from build123d import *

# Parameters (mm, degrees)
FORK_BOSS_15MM_DEPTH           = 15
SKETCH1_10_R                   = 11.5
SKETCH1_10_R_2                 = 4.5
PLATE_BOSS_12MM_DEPTH          = 12
POCKET_START                   = -7
POCKET_AND_HOLES_CUT_7MM_DEPTH = 7


with BuildPart() as part:
    # Bracket Outline Sketch → Fork Boss 15mm (new body)
    with BuildSketch(Plane.XY):
        with BuildLine():
            Line((-17.348851567, 85.016364122), (17.292164585, 65.016364122))
            ThreePointArc((17.292164585, 65.016364122), (21.08625981, 64.51686201), (24.122291604, 66.846491141))
            Line((24.122291604, 66.846491141), (29.979005279, 76.990616791))
            Line((29.979005279, 76.990616791), (39.122291604, 92.827253255))
            Line((39.122291604, 92.827253255), (30.490381057, 97.810889132))
            Line((30.490381057, 97.810889132), (17.990381057, 76.160254038))
            Line((17.990381057, 76.160254038), (-7.990381057, 91.160254038))
            Line((-7.990381057, 91.160254038), (4.509618943, 112.810889132))
            Line((4.509618943, 112.810889132), (-4.178978585, 117.827253255))
            Line((-4.178978585, 117.827253255), (-19.178978585, 91.846491141))
            ThreePointArc((-19.178978585, 91.846491141), (-19.678480698, 88.052395915), (-17.348851567, 85.016364122))
        make_face()
    extrude(amount=FORK_BOSS_15MM_DEPTH)

    # Sketch1_10 → Plate Boss 12mm (add)
    with BuildSketch(Plane.XY):
        with BuildLine():
            ThreePointArc((24.122291604, 66.846491141), (21.08625981, 64.51686201), (17.292164585, 65.016364122))
            Line((17.292164585, 65.016364122), (-17.348851567, 85.016364122))
            ThreePointArc((-17.348851567, 85.016364122), (-19.678480698, 88.052395915), (-19.178978585, 91.846491141))
            Line((-19.178978585, 91.846491141), (-22.741186866, 85.676565412))
            ThreePointArc((-22.741186866, 85.676565412), (-25.323096431, 80.149782404), (-26.906195607, 74.258654802))
            Line((-26.906195607, 74.258654802), (-38.965270802, 5.868240888))
            ThreePointArc((-38.965270802, 5.868240888), (-37.871454253, 1.786061952), (-34.041232037, 0))
            Line((-34.041232037, 0), (34.041232037, 0))
            ThreePointArc((34.041232037, 0), (37.871454253, 1.786061952), (38.965270802, 5.868240888))
            Line((38.965270802, 5.868240888), (28.201741138, 66.911250985))
            ThreePointArc((28.201741138, 66.911250985), (28.201741138, 72.107623698), (29.979005279, 76.990616791))
            Line((29.979005279, 76.990616791), (24.122291604, 66.846491141))
        make_face()
        with Locations((0, 20)):
            Circle(SKETCH1_10_R, mode=Mode.SUBTRACT)
        with Locations((0, 45)):
            Circle(SKETCH1_10_R_2, mode=Mode.SUBTRACT)
    extrude(amount=PLATE_BOSS_12MM_DEPTH)

    # Pocket and Holes Sketch → Pocket and Holes Cut 7mm (cut)
    with BuildSketch(Plane.XY.offset(12).offset(POCKET_START)):
        with BuildLine():
            Line((25.009745942, 68.383607145), (24.122291604, 66.846491141))
            ThreePointArc((24.122291604, 66.846491141), (21.08625981, 64.51686201), (17.292164585, 65.016364122))
            Line((17.292164585, 65.016364122), (-17.348851567, 85.016364122))
            ThreePointArc((-17.348851567, 85.016364122), (-18.180803852, 85.618476392), (-18.872189895, 86.377863731))
            Line((-18.872189895, 86.377863731), (-20.143109976, 84.176565019))
            ThreePointArc((-20.143109976, 84.176565019), (-22.504396013, 79.122684974), (-23.952156408, 73.735536834))
            Line((-23.952156408, 73.735536834), (-36.010847543, 5.347296355))
            ThreePointArc((-36.010847543, 5.347296355), (-35.573320923, 3.714424781), (-34.041232037, 3))
            Line((-34.041232037, 3), (34.041232037, 3))
            ThreePointArc((34.041232037, 3), (35.573320923, 3.714424781), (36.010847543, 5.347296355))
            Line((36.010847543, 5.347296355), (25.247317879, 66.390306452))
            ThreePointArc((25.247317879, 66.390306452), (25.100664631, 67.383635431), (25.009745942, 68.383607145))
        make_face()
    extrude(amount=POCKET_AND_HOLES_CUT_7MM_DEPTH, mode=Mode.SUBTRACT)


solid = part.part
For this review, take the finished solid that the model builds, in its own axes (mm). A direction names the side the tool comes from. Round coordinates to 2 decimals unless told otherwise and drop trailing zeros. Order: outer loops, then holes, each group sorted by start corner. A loop starts at its lowest first (then second) coordinate and runs counter-clockwise, first axis right, second up. Notation, with made-up numbers: (85, 46.25) -> (111, 46.25) arc R19 ccw to (111, 81.25) -> close; hole circle Ø2 at (37.5, -31). An arc over 180 degrees is marked (long way). Write item = value, one per line. Start each with the question number.
1) The part is to be moulded in two halves that separate along X. For faces 1 (the face through (8, 47, 0)), 2 (the face through (-1.83, 101.83, 7.4)), 3 (the face through (-25.294, 80.23, 5.916)), 4 (the face through (33.66, 35.96, 5.92)), say which applies: +X half, -X half, draft (parallel to the pull), parting line (faces both ways), or undercut.
2) To check wall thickness, follow line 1 (Y direction, x = -4.5, z = 5.25); line 2 (Y direction, x = 0, z = 2.7); line 3 (X direction, y = 79.5, z = 5.5). State the ranges of each line that lie inside material, in increasing order. Write a range as from..to.
3) Tool access review of faces 5 (the face through (34.867, 95.284, 7.395)), 6 (the face through (-29.9, 40, 8.5)), 7 (the face through (5.182, 83.555, 7.395)): name each direction out of +Z, -Z, +X, -X, +Y, -Y from which nothing blocks a thin tool from reaching the whole face with its end or side.
4) Insertion check: pin 1 (1.5 mm diameter, centred on y = 21.5, z = 9.5, fed in from +X); pin 2 (1.5 mm diameter, centred on x = 10.5, z = 13.5, fed in from +Y); pin 3 (8 mm diameter, centred on x = -23, z = 2, fed in from +Y). Each pin has a flat end and moves straight along its axis. Give the tip position at first contact, or say it passes through.
5) Take a section at D-D on y = 45. State the section outline as (x, z) points, plus the area to 3 significant figures.
6) Take a section at B-B on z = 1.75. State the section outline as (x, y) points, plus the area to 3 significant figures.
7) Take a section at A-A on z = 8.5. State the section outline as (x, y) points.
8) Take a section at C-C on x = 0. State the section outline as (y, z) points.
Verdict:
q1.face_1 = draft
q1.face_2 = undercut
q1.face_3 = -X half
q1.face_4 = +X half
q2.line_1 = 0..3, 77.6..89.15, 97.21..117.27
q2.line_2 = 0..8.5, 31.5..40.5, 49.5..86.55, 105..115.41
q2.line_3 = -25.55..-22.36, -7.79..12.21, 19.92..31.43
q3.face_5 = +Z, -Z, +X, +Y
q3.face_6 = +Z
q3.face_7 = +Z, -Z
q4.pin_1 = 36.34
q4.pin_2 = 80.92
q4.pin_3 = 92.16
q5.outline = (-32.07, 0) -> (-4.5, 0) -> (-4.5, 5) -> (-29.02, 5) -> (-29.02, 12) -> (-32.07, 12) -> close; (4.5, 0) -> (32.07, 0) -> (32.07, 12) -> (29.02, 12) -> (29.02, 5) -> (4.5, 5) -> close
q5.area = 318 mm2
q6.outline = (-38.97, 5.87) arc R5 ccw to (-34.04, 0) -> (34.04, 0) arc R5 ccw to (38.97, 5.87) -> (28.2, 66.91) arc R14.96 cw to (29.98, 76.99) -> (39.12, 92.83) -> (30.49, 97.81) -> (17.99, 76.16) -> (-7.99, 91.16) -> (4.51, 112.81) -> (-4.18, 117.83) -> (-22.74, 85.68) arc R35 ccw to (-26.91, 74.26) -> close; hole circle Ø23 at (0, 20); hole circle Ø9 at (0, 45)
q6.area = 5,510 mm2
q7.outline = (-38.97, 5.87) arc R5 ccw to (-34.04, 0) -> (34.04, 0) arc R5 ccw to (38.97, 5.87) -> (28.2, 66.91) arc R14.96 cw to (29.98, 76.99) -> (39.12, 92.83) -> (30.49, 97.81) -> (17.99, 76.16) -> (-7.99, 91.16) -> (4.51, 112.81) -> (-4.18, 117.83) -> (-22.74, 85.68) arc R35 ccw to (-26.91, 74.26) -> close; hole (-36.01, 5.35) arc R2 ccw to (-34.04, 3) -> (34.04, 3) arc R2 ccw to (36.01, 5.35) -> (25.25, 66.39) arc R17.96 cw to (25.01, 68.38) -> (24.12, 66.85) arc R5 cw to (17.29, 65.02) -> (-17.35, 85.02) arc R5 cw to (-18.87, 86.38) -> (-20.14, 84.18) arc R32 ccw to (-23.95, 73.74) -> close
q8.outline = (0, 0) -> (8.5, 0) -> (8.5, 5) -> (3, 5) -> (3, 12) -> (0, 12) -> close; (31.5, 0) -> (40.5, 0) -> (40.5, 5) -> (31.5, 5) -> close; (49.5, 0) -> (86.55, 0) -> (86.55, 15) -> (75, 15) -> (75, 5) -> (49.5, 5) -> close; (105, 0) -> (115.41, 0) -> (115.41, 15) -> (105, 15) -> close
